Input: part model. Units: mm. Frame: model coordinates. Give positions to 0.01 mm unless a question says otherwise; leave off trailing zeros. Write each loop counter-clockwise with the first axis right and the second up, starting at its lowest first coordinate (ties: lowest second). Pieces come first, ordered by that corner, then holes. Notation, with made-up numbers: (38, 76.25) - (58, 76.25) arc R22 cw to (58, 87.25) - close; hole circle Ø4 at (83, 59). An arc over 180 degrees is marked (long way). Answer as CSV lines item,"result". Start each with the question number.
from build123d import *

# Parameters (mm, degrees)
EXTRUDE_1_DEPTH = 7
CHAMFER_1_SIZE  = 0.4


with BuildPart() as part:
    # 草图1 → 凸台-拉伸1 (new body)
    with BuildSketch(Plane(origin=(0, 0, 0), x_dir=(1, 0, 0), z_dir=(0, 1, 0))):
        with BuildLine():
            Line((3.5, 0), (32, 0))
            Line((32, 0), (32, -7))
            Line((32, -7), (3.5, -7))
            ThreePointArc((3.5, -7), (0, -3.5), (3.5, 0))
        make_face()
    extrude(amount=EXTRUDE_1_DEPTH)

    # 倒角1
    chamfer_1_edges = [part.edges().sort_by_distance(p)[0] for p in [
        (32, 7, 3.5),
        (17.75, 7, 0),
        (0, 7, 3.5),
        (17.75, 0, 0),
        (32, 0, 3.5),
        (17.75, 0, 7),
        (0, 0, 3.5),
        (17.75, 7, 7),
    ]]
    chamfer(chamfer_1_edges, length=CHAMFER_1_SIZE)


solid = part.part
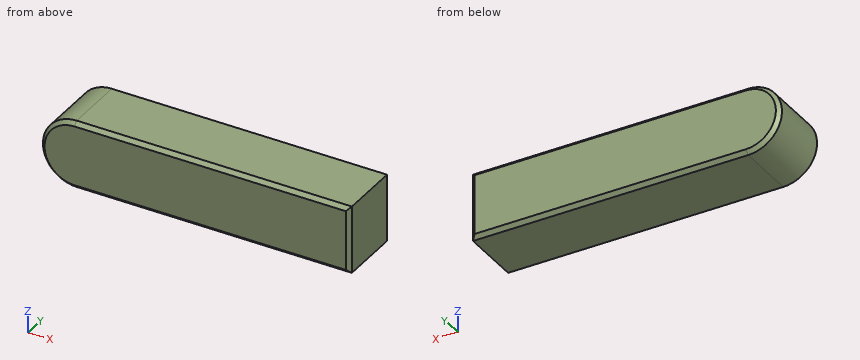
1) Material intervals for line 1 (X direction, y = 2, z = 4.25); line 2 (X direction, y = 4, z = 6.5); line 3 (Z direction, x = 2.5, y = 2.25), sorted ascending. Write a range as from..to.
2) Cut plane A-A on y = 4.5. Output: boundary loops of the cut face in (x, z), and give its area (3 significant figures).
3) Contact query for a flat-ended pin moving along its axis: P1, Ø4, axis at y = 5, z = 3, coming from the -X side. Output: stop coordinate, or through.
Numbers:
1,line 1,"x = 0.08..32"
1,line 2,"x = 1.7..32"
1,line 3,"z = 0.15..6.85"
2,outline,"(3.5, 0) - (32, 0) - (32, 7) - (3.5, 7) arc R3.5 ccw to start"
2,area,"219 mm²"
3,P1,"stops at x = 0"
